For this review, take the finished solid that the model builds, in its own axes (mm). Face numbers are marked on the shaded views. A direction names the side the tool comes from. Give positions to 0.01 mm unless a question says otherwise; leave off trailing zeros. Write each loop counter-clockwise with the first axis right and the second up, starting at its lowest first coordinate (ties: lowest second). Pieces come first, ordered by that corner, then holes.
Q1. Machinability: for the marked faces 5 and 6, which of the approach directions +Z, -Z, +X, -X, +Y, -Y give a long, thin tool a straight path to every point of the face, cutting with its end or side? Answer none if there is none.
Q2. For line 1 (X direction, y = -20.5, z = 1); line 2 (X direction, y = 34.5, z = 0.75); line 3 (Y direction, x = 85, z = 10), list the stretches that pass through material, from the lowest coordinate up.
Q3. We need section A-A (y = -35). Write out the cut boundary in (x, z), then the cut area to 3 significant figures.
Q4. We need section C-C (x = 53.5). Write out the cut boundary in (y, z), then the cut area to 3 significant figures.
Q5. We need section D-D (y = 0). Write out the cut boundary in (x, z), then the cut area to 3 significant figures.
Q6. We need section B-B (z = 4). Give the number of separate pieces and of enclosed holes in the cut face, then the cut area to 3 significant figures.
Q7. Mouldability with a two-part tool opening along Y and no side actions: class the marked faces 1, 2, 3 and 4 as released by +Y, released by -Y, zero draft, split by the parting line, or undercut.
Q8. Insertion check: P1, Ø10.5, axis at x = 15.8, y = -20, coming from the -Z side. The pin has a flat end and moves straight along its axis. Give the tip position at first contact, or say it passes through.
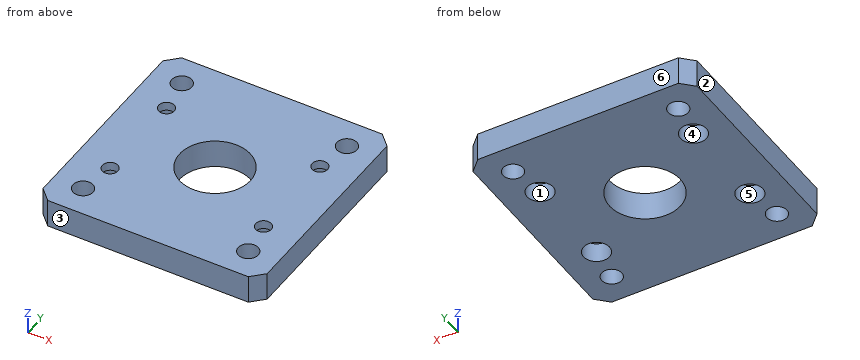
```python
from build123d import *

# Parameters (mm, degrees)
SKETCH_1_W                = 95
SKETCH_1_H                = 95
EXTRUDE_1_DEPTH           = 12
SKETCH_2_R                = 15
CUT_EXTRUDE_1_DEPTH       = 108.604604424
HOLE_WIZARD_1_D           = 6.6
HOLE_WIZARD_1_CBORE_D     = 11
HOLE_WIZARD_1_CBORE_DEPTH = 8.3
HOLE_WIZARD_M10_2_D       = 8.5
CHAMFER_1_SIZE            = 5


with BuildPart() as part:
    # 草图1 → 凸台-拉伸1 (new body)
    with BuildSketch(Plane.XY):
        with Locations((48.304493075, 0)):
            Rectangle(SKETCH_1_W, SKETCH_1_H)
    extrude(amount=EXTRUDE_1_DEPTH)

    # 草图2 → 切除-拉伸1 (cut, through all)
    with BuildSketch(Plane.XY.offset(12)):
        with Locations((48.304493075, 0)):
            Circle(SKETCH_2_R)
    extrude(amount=-CUT_EXTRUDE_1_DEPTH, mode=Mode.SUBTRACT)

    # 打孔尺寸(%根据)内六角圆柱头螺钉的类型1 (through all)
    with Locations(Plane(origin=(80.804493075, 20, 0), x_dir=(-1, 0, 0), z_dir=(0, 0, -1))):
        with Locations((0, 0), (65, 0), (65, -40), (0, -40)):
            CounterBoreHole(HOLE_WIZARD_1_D / 2, HOLE_WIZARD_1_CBORE_D / 2, HOLE_WIZARD_1_CBORE_DEPTH)

    # M10 螺纹孔2 (through all)
    with Locations(Plane(origin=(83.304493075, 35, 0), x_dir=(-1, 0, 0), z_dir=(0, 0, -1))):
        with Locations((0, 0), (70, 0), (70, -70), (0, -70)):
            Hole(HOLE_WIZARD_M10_2_D / 2)

    # 倒角1
    chamfer_1_edges = [part.edges().sort_by_distance(p)[0] for p in [
        (0.804493075, 47.5, 6),
        (95.804493075, 47.5, 6),
        (95.804493075, -47.5, 6),
        (0.804493075, -47.5, 6),
    ]]
    chamfer(chamfer_1_edges, length=CHAMFER_1_SIZE)


solid = part.part
```
Computed:
1. face 5: -Z
1. face 6: +Z, -Z, +X, -X, +Y
2. line 1: x = 0.8 to 10.33, 21.28 to 75.33, 86.28 to 95.8
2. line 2: x = 0.8 to 9.08, 17.52 to 79.08, 87.52 to 95.8
2. line 3: y = -47.5 to -38.9, -31.1 to 31.1, 38.9 to 47.5
3. outline: (0.8, 0) - (9.05, 0) - (9.05, 12) - (0.8, 12) - close; (17.55, 0) - (79.05, 0) - (79.05, 12) - (17.55, 12) - close; (87.55, 0) - (95.8, 0) - (95.8, 12) - (87.55, 12) - close
3. area: 936 mm2
4. outline: (-47.5, 0) - (-14.07, 0) - (-14.07, 12) - (-47.5, 12) - close; (14.07, 0) - (47.5, 0) - (47.5, 12) - (14.07, 12) - close
4. area: 802 mm2
5. outline: (0.8, 0) - (33.3, 0) - (33.3, 12) - (0.8, 12) - close; (63.3, 0) - (95.8, 0) - (95.8, 12) - (63.3, 12) - close
5. area: 780 mm2
6. separate pieces: 1
6. enclosed holes: 9
6. area: 7,660 mm2
7. face 1: undercut
7. face 2: zero draft
7. face 3: released by -Y
7. face 4: undercut
8. P1: stops at z = 8.3
